from build123d import *

# Parameters (mm, degrees)
SKETCH_1_W                  = 135
SKETCH_1_H                  = 605
EXTRUDE_1_DEPTH             = 6
HOLE_WIZARD_M6_1_D          = 5
HOLE_WIZARD_M6_1_DEPTH      = 17
HOLE_WIZARD_M6_1_TIP        = 1.502151548
HOLE_WIZARD_2_D             = 6.6
HOLE_WIZARD_2_CBORE_D       = 11
HOLE_WIZARD_2_CBORE_DEPTH   = 6.8
HOLE_WIZARD_2_2_D           = 6.6
HOLE_WIZARD_2_2_CBORE_D     = 11
HOLE_WIZARD_2_2_CBORE_DEPTH = 6.8


with BuildPart() as part:
    # 草图1 → 凸台-拉伸1 (new, symmetric)
    with BuildSketch(Plane.XY):
        Rectangle(SKETCH_1_W, SKETCH_1_H)
    extrude(amount=EXTRUDE_1_DEPTH, both=True)

    # M6 螺纹孔1
    with Locations(Plane(origin=(0, 302.5, 0), x_dir=(1, 0, 0), z_dir=(0, 1, 0))):
        with Locations((50, 0), (-30, 0), (30, 0), (-405, -6), (-50, 0)):
            Hole(HOLE_WIZARD_M6_1_D / 2, depth=HOLE_WIZARD_M6_1_DEPTH)
            with Locations((0, 0, -(HOLE_WIZARD_M6_1_DEPTH + HOLE_WIZARD_M6_1_TIP / 2))):  # 118° drill point
                Cone(0, HOLE_WIZARD_M6_1_D / 2, HOLE_WIZARD_M6_1_TIP, mode=Mode.SUBTRACT)

    # Hole Wizard 2 (through all)
    with Locations(Plane(origin=(0, 0, -6), x_dir=(-1, 0, 0), z_dir=(0, 0, -1))):
        with Locations((-60, 290.5), (60, 290.5), (-60, 274.5), (60, 274.5)):
            CounterBoreHole(HOLE_WIZARD_2_D / 2, HOLE_WIZARD_2_CBORE_D / 2, HOLE_WIZARD_2_CBORE_DEPTH)

    # Hole Wizard 2 2 (through all)
    with Locations(Plane(origin=(0, 0, -6), x_dir=(-1, 0, 0), z_dir=(0, 0, -1))):
        with Locations((-32.5, -153.5), (-32.5, -228.5), (32.5, -228.5), (32.5, -153.5), (32.5, -173.5), (32.5, -248.5), (-32.5, -248.5), (-32.5, -173.5), (32.5, -268.5), (32.5, -193.5), (-32.5, -193.5), (-32.5, -268.5)):
            CounterBoreHole(HOLE_WIZARD_2_2_D / 2, HOLE_WIZARD_2_2_CBORE_D / 2, HOLE_WIZARD_2_2_CBORE_DEPTH)


solid = part.part
The model under review builds one solid part; all positions refer to its coordinate system, in mm. Coordinates: 2 decimals unless noted, no trailing zeros. Put each result on its own line as item: value.
1) Clearance check with a flat-ended pin moving along its axis: pin 1 Ø10.5 at (x, y) = (60, 274.5) entering from -Z. State where the tip first meets the part, or that it passes through.
Computed:
pin 1: stops at z = 0.8
2) Draft analysis for pull direction Y (two halves, no side actions). For faces 1 (the flat face through (-1, -302.5, 0)), 2 (the flat face through (-35, -231, 0.8)), 3 (the flat face through (-1, 4, -6)), state which applies: released by +Y, released by -Y, zero draft, split by the parting line, or undercut.
Computed:
face 1: released by -Y
face 2: undercut
face 3: zero draft
3) Wall thickness on probe 1 along X at (y, z) = (-193.5, 4.45); probe 2 along X at (y, z) = (290.5, 4.2); probe 3 along Z at (x, y) = (50, 297): over which ranges is each line inside the solid? List them lowest first. Write a range as [from, to].
Computed:
probe 1: x = [-67.5, -35.8], [-29.2, 29.2], [35.8, 67.5]
probe 2: x = [-67.5, -63.3], [-56.7, 56.7], [63.3, 67.5]
probe 3: z = [-6, -2.5], [2.5, 6]
